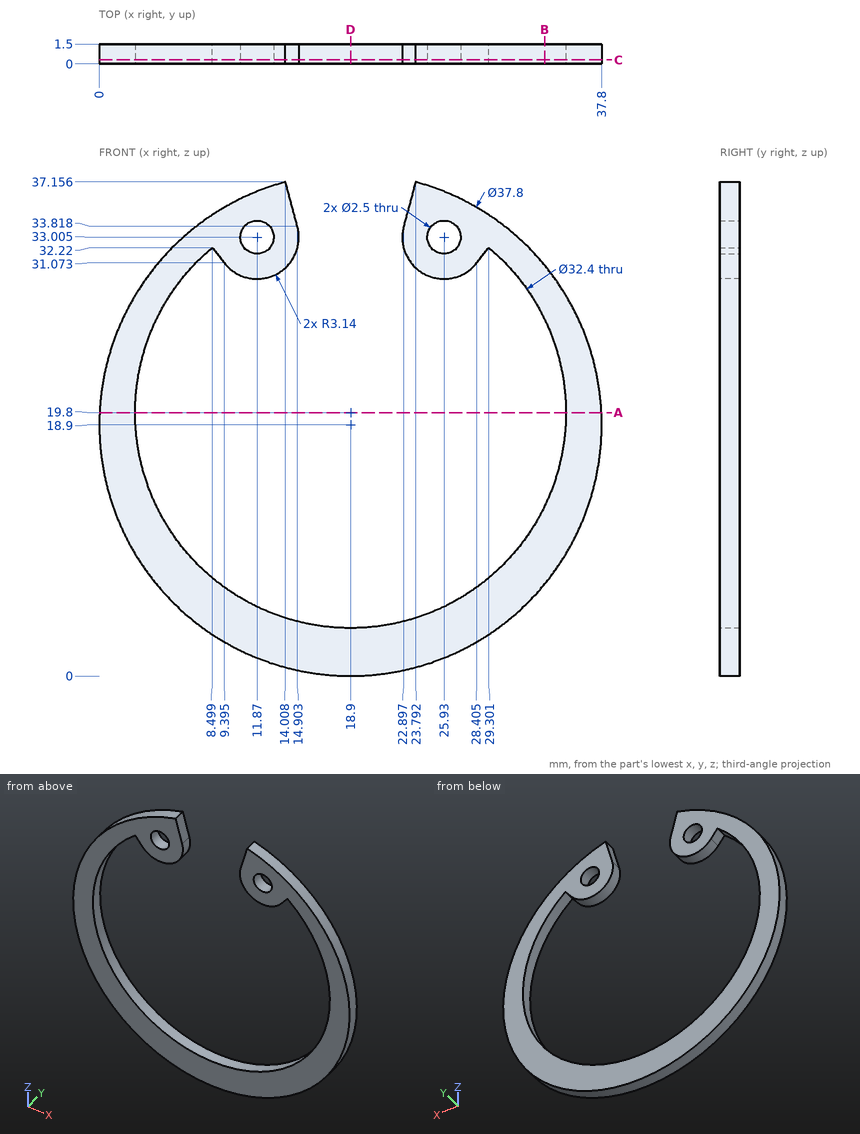
Job drawing, mm, ordinate dimensions from the low corner. One solid piece. Coordinates: 2 decimals unless noted, no trailing zeros. Order: outer loops, then holes, each group sorted by start corner. A loop starts at its lowest first (then second) coordinate and runs counter-clockwise, first axis right, second up. Notation, with made-up numbers: (-31, 84) - (23, 84) arc R29 ccw to (23, 120) - close; hole circle Ø3 at (55.25, 80). An arc over 180 degrees is marked (long way). Write each question's results on one line, items separated by ' | '. Start each with the question number.
Item 1: Band-saw the part on A-A on z = 19.8. Write the cut outline in (x, y).
Item 2: Band-saw the part on C-C on y = 0.3. State how many separate pieces and enclosed holes the cut face has, and give its area (3 significant figures).
Item 3: Band-saw the part on B-B on x = 33.5. Write the cut outline in (y, z).
Item 4: Wall check: probe 1 along X at (y, z) = (0.3, 33.5) (1 decimal); probe 2 along Z at (x, y) = (4.5, 0.9) (1 decimal); probe 3 along Z at (x, y) = (10.5, 0.6). Give the ranges that are in metal, low to high. Write a range as [from, to].
Item 5: Flat gauge pin, fed straight in: pin 1 (4 mm diameter, centred on x = 25.93, z = 33.01, fed in from -Y). Where does the tip first touch, or does it go through?
Item 6: Band-saw the part on D-D on x = 18.9. Write the cut outline in (y, z).
Numbers:
1) outline: (0.02, 0) - (2.7, 0) - (2.7, 1.5) - (0.02, 1.5) - close; (35.1, 0) - (37.78, 0) - (37.78, 1.5) - (35.1, 1.5) - close
2) separate pieces: 1 | enclosed holes: 2 | area: 317 mm^2
3) outline: (0, 6.9) - (1.5, 6.9) - (1.5, 12.78) - (0, 12.78) - close; (0, 26.82) - (1.5, 26.82) - (1.5, 30.9) - (0, 30.9) - close
4) probe 1: [6.9, 10.7], [13, 15], [22.8, 24.8], [27.1, 30.9] | probe 2: [6.7, 12.4], [27.2, 31.1] | probe 3: [1.97, 5.95], [30.18, 35.83]
5) pin 1: y = 0
6) outline: (0, 0) - (1.5, 0) - (1.5, 3.6) - (0, 3.6) - close
